Build history of the part. All positions in model axes, mm. A direction names the side the tool comes from. Coordinates: 2 decimals unless noted, no trailing zeros. Write each loop counter-clockwise with the first axis right and the second up, starting at its lowest first coordinate (ties: lowest second). Pieces come first, ordered by that corner, then holes. Notation, with made-up numbers: (-24.5, 74) -> (18.5, 74) arc R30 cw to (18.5, 113) -> close; hole circle Ø2 at (-20.75, 70.25). An arc over 180 degrees is marked (long way). Write each question's results on one line, items separated by ' | '. Start each with the question number.
Q1. Two-plate mould, pull along X, no slides. Class faces 1 (the face through (-0.35, 0.11, -36.56)), 2 (the face through (-2, -2, 50)), 3 (the face through (5, 0, 1)), 4 (the face through (0.27, -0.2, 36.54)): released by +X, released by -X, zero draft, split by the parting line, or undercut.
Q2. Saw through at B-B on z = -12. Give the cut face in (x, y).
Q3. Tool access for faces 5 (the face through (-2.003, 0.631, -43.887)), 6 (the face through (-2.003, 0.631, 43.713)), 7 (the face through (2, -2, -50)): list every direction of +Z, -Z, +X, -X, +Y, -Y with a clear straight run to the whole face (end or side of a thin tool).
Q4. Saw through at A-A on z = 43.5. Give the cut face in (x, y).
Q5. Drill centre lines: line 1 (Y direction, x = 0, z = -45.75); line 2 (X direction, y = -0.25, z = -25); line 3 (Y direction, x = 3, z = 25). Where is each one in solid material? Low to high.
Q6. Drop flat-ended pins along their axis: pin 1 Ø3.5 at (x, y) = (0, 0) entering from -Z; pin 2 Ø2 at (x, z) = (-1.5, -14.5) entering from -Y; pin 3 Ø1.5 at (y, z) = (3.5, 38.5) entering from -X. Give the stop position or say it passes through.
from build123d import *


with BuildPart() as part:
    # 草图1 → 旋转1 (revolve)
    with BuildSketch(Plane.XZ, mode=Mode.PRIVATE) as revolve_1_sk:
        Polygon((2.1, 37.6), (0, 36.3381927), (0, -36.3381927), (2.1, -37.6), (2.1, -50), (4, -50), (5, -49), (5, 49), (4, 50), (2.1, 50), align=None)
    revolve(revolve_1_sk.sketch.rotate(Axis((0, 0, 50), (0, 0, -1)), 180), axis=Axis((0, 0, 50), (0, 0, -1)))


solid = part.part
Returned:
1) face 1: undercut | face 2: zero draft | face 3: split by the parting line | face 4: undercut
2) outline: circle Ø10 at (0, 0)
3) face 5: -Z | face 6: +Z | face 7: -Z, +X, -X, +Y, -Y
4) outline: circle Ø10 at (0, 0); hole circle Ø4.2 at (0, 0)
5) line 1: y = -5 to -2.1, 2.1 to 5 | line 2: x = -4.99 to 4.99 | line 3: y = -4 to 4
6) pin 1: stops at z = -37.39 | pin 2: stops at y = -4.97 | pin 3: stops at x = -4.18
